```python
from build123d import *

# Parameters (mm, degrees)
BOSS_EXTRUDE1_DEPTH = 30


with BuildPart() as part:
    # Sketch1 → Boss-Extrude1 (new body)
    with BuildSketch(Plane.XY):
        with BuildLine():
            Line((110, 0), (110, 40))
            ThreePointArc((110, 40), (135, 65), (160, 40))
            Line((160, 40), (160, 0))
            Line((160, 0), (270, 0))
            Line((270, 0), (270, 482))
            Line((270, 482), (260, 492))
            Line((260, 492), (10, 492))
            Line((10, 492), (0, 482))
            Line((0, 482), (0, 0))
            Line((0, 0), (110, 0))
        make_face()
    extrude(amount=BOSS_EXTRUDE1_DEPTH)


solid = part.part
```
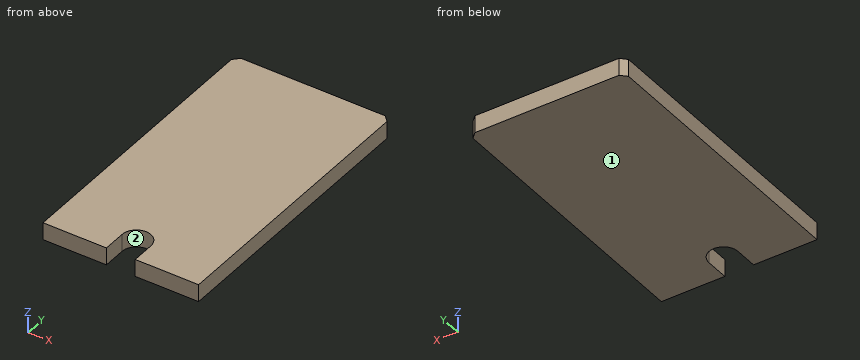
CAD build for the part. Positions are in the model's coordinates, mm. Face numbers are marked on the shaded views. Round coordinates to 2 decimals unless told otherwise and drop trailing zeros. Loops run counter-clockwise (first coordinate to the right, second up) from the corner with the lowest first, then second, coordinate; pieces in that order, holes last. Notation, with made-up numbers: (14, -10) - (58, -10) arc R15 ccw to (58, 10) - close; hole circle Ø7 at (52.5, -28.5). An arc over 180 degrees is marked (long way). Return JSON: item names as keys, results as strings. Group by question number.
Q1. Band-saw the part on A-A on z = 12.75. Give the cut face in (x, y), plus the area to 3 significant figures.
Q2. Band-saw the part on B-B on x = 135. Give the cut face in (y, z), plus the area to 3 significant figures.
Q3. Drill centre lines: line 1 along X through (y, z) = (39, 19.5); line 2 along X through (y, z) = (59, 13.25); line 3 along Y through (x, z) = (125, 11). Where is each one in solid material? Low to high. Write a range as [from, to].
Q4. Two-plate mould, pull along X, no slides. Class the marked faces 1 and 2: +X half, -X half, draft (parallel to the pull), parting line (faces both ways), or undercut.
Solutions:
{
 "1": {"outline": "(0, 0) - (110, 0) - (110, 40) arc R25 cw to (160, 40) - (160, 0) - (270, 0) - (270, 482) - (260, 492) - (10, 492) - (0, 482) - close", "area": "130,000 mm^2"},
 "2": {"outline": "(65, 0) - (492, 0) - (492, 30) - (65, 30) - close", "area": "12,800 mm^2"},
 "3": {"line 1": "x = [0, 110], [160, 270]", "line 2": "x = [0, 118.75], [151.25, 270]", "line 3": "y = [62.91, 492]"},
 "4": {"face 1": "draft", "face 2": "undercut"}
}
